The listing builds one solid part. Answer for the finished solid, in the listing's coordinates (mm). Face numbers are marked on the shaded views. Give positions to 0.01 mm unless a question says otherwise; leave off trailing zeros. Write each loop counter-clockwise with the first axis right and the second up, starting at its lowest first coordinate (ties: lowest second). Pieces come first, ordered by that corner, then holes. Notation, with made-up numbers: M -26.75,-27.5 L 29.25,-27.5 A9 ccw 29.25,-10.5 Z; hole C 10,10.25 d10. An arc over 180 degrees is marked long. Answer as a JSON object with one key per item and string values.
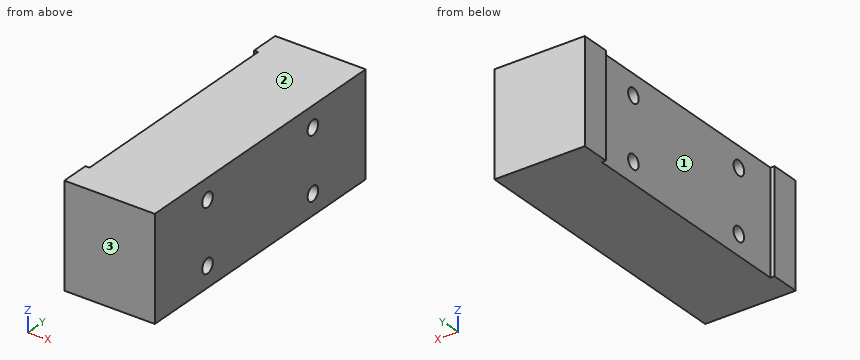
```python
from build123d import *

# Parameters (mm, degrees)
SKETCH1_W           = 22
SKETCH1_H           = 25
BOSS_EXTRUDE1_DEPTH = 70
SKETCH2_R           = 1.75
CUT_EXTRUDE1_DEPTH  = 75.432855649
SKETCH4_W           = 25
SKETCH4_H           = 56
CUT_EXTRUDE3_DEPTH  = 1


with BuildPart() as part:
    # Sketch1 → Boss-Extrude1 (new body)
    with BuildSketch(Plane(origin=(0, 0, 0), x_dir=(1, 0, 0), z_dir=(0, 1, 0))):
        Rectangle(SKETCH1_W, SKETCH1_H)
    extrude(amount=BOSS_EXTRUDE1_DEPTH)

    # Sketch2 → Cut-Extrude1 (cut, through all)
    with BuildSketch(Plane(origin=(11, 0, 0), x_dir=(0, 0, -1), z_dir=(1, 0, 0))):
        with Locations((-7.5, 52.5)):
            Circle(SKETCH2_R)
        with Locations(Location((7.5, 52.5, 0), (0, 0, 180))):
            Circle(SKETCH2_R)
        with Locations((7.5, 17.5)):
            Circle(SKETCH2_R)
        with Locations(Location((-7.5, 17.5, 0), (0, 0, 180))):
            Circle(SKETCH2_R)
    extrude(amount=-CUT_EXTRUDE1_DEPTH, mode=Mode.SUBTRACT)

    # Sketch4 → Cut-Extrude3 (cut)
    with BuildSketch(Plane.ZY.offset(11)):
        with Locations((0, 35)):
            Rectangle(SKETCH4_W, SKETCH4_H)
    extrude(amount=-CUT_EXTRUDE3_DEPTH, mode=Mode.SUBTRACT)


solid = part.part
```
1. The mould has two halves that part along Y. Classify the marked faces 1, 2 and 3: released by +Y, released by -Y, zero draft, split by the parting line, or undercut.
Verdict:
{"face 1": "undercut", "face 2": "zero draft", "face 3": "released by -Y"}
2. A cutting plane is placed at A-A, the plane y = 17.5. Give the vertices of the cut face in (x, z), plus the area to 3 significant figures.
Verdict:
{"outline": "M -10,-12.5 L 11,-12.5 L 11,-9.25 L -10,-9.25 Z; M -10,-5.75 L 11,-5.75 L 11,5.75 L -10,5.75 Z; M -10,9.25 L 11,9.25 L 11,12.5 L -10,12.5 Z", "area": "378 mm2"}
3. A cutting plane is placed at D-D, the plane z = -10. Give the vertices of the cut face in (x, y), plus the area to 3 significant figures.
Verdict:
{"outline": "M -11,0 L 11,0 L 11,70 L -11,70 L -11,63 L -10,63 L -10,7 L -11,7 Z", "area": "1,480 mm2"}
4. A cutting plane is placed at C-C, the plane x = 1.75. Give the vertices of the cut face in (y, z), plus the area to 3 significant figures.
Verdict:
{"outline": "M 0,-12.5 L 70,-12.5 L 70,12.5 L 0,12.5 Z; hole C 17.5,-7.5 d3.5; hole C 17.5,7.5 d3.5; hole C 52.5,-7.5 d3.5; hole C 52.5,7.5 d3.5", "area": "1,710 mm2"}
5. A cutting plane is placed at B-B, the plane z = 7.5. Give the vertices of the cut face in (x, y).
Verdict:
{"outline": "M -11,0 L 11,0 L 11,15.75 L -10,15.75 L -10,7 L -11,7 Z; M -11,63 L -10,63 L -10,54.25 L 11,54.25 L 11,70 L -11,70 Z; M -10,19.25 L 11,19.25 L 11,50.75 L -10,50.75 Z"}
6. Consider line 1 along Y through (x, z) = (-0.25, 7.5); line 2 along Z through (x, y) = (-2.5, 53); line 3 along Y through (x, z) = (6, -6.5). Determine where each line is inside the solid, lowest interval first.
Verdict:
{"line 1": "y = 0 to 15.75, 19.25 to 50.75, 54.25 to 70", "line 2": "z = -12.5 to -9.18, -5.82 to 5.82, 9.18 to 12.5", "line 3": "y = 0 to 16.06, 18.94 to 51.06, 53.94 to 70"}
7. Flat-ended cylindrical pins translate along their axes: pin 1 (10 mm diameter, centred on x = 5, z = 2.5, fed in from -Y); pin 2 (10 mm diameter, centred on y = 57, z = -10, fed in from -X). Find the tip coordinate at first contact, or state that the pin passes through.
Verdict:
{"pin 1": "stops at y = 0", "pin 2": "stops at x = -10"}
